Study the drawing (mm; zero at the part's minimum x, y, z) and answer. A direction names the side the tool comes from. Give positions to 0.01 mm unless a question says otherwise; leave off trailing zeros. Loops run counter-clockwise (first coordinate to the right, second up) from the corner with the lowest first, then second, coordinate; pieces in that order, holes last. Notation, with made-up numbers: M 67.5,30 L 86.5,30 A24 ccw 86.5,62 Z; hole C 25,16 d7. An arc over 180 degrees is marked long. Return JSON: item names as keys, results as strings.
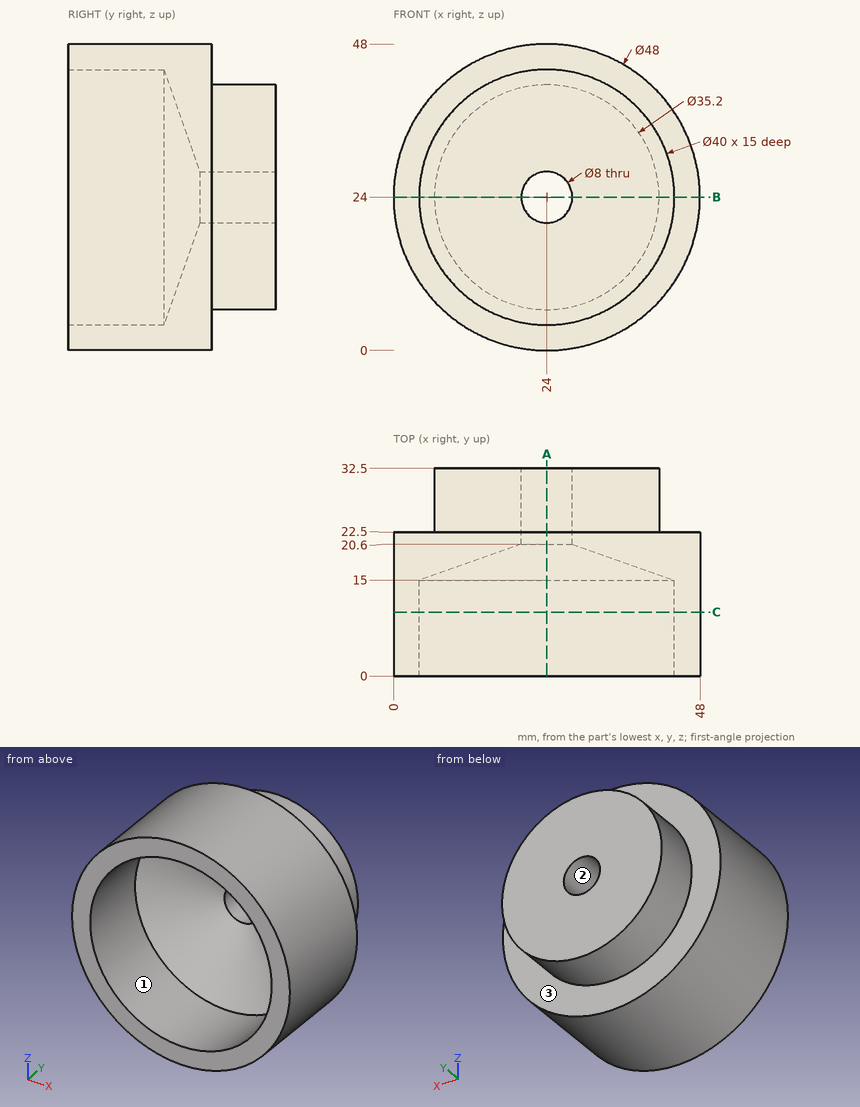
(1) The part is cut by section B-B (z = 24). Determine the outline of the cut face in (x, y), and give its area (3 significant figures).
Values follow:
{"outline": "M 0,0 L 4,0 L 4,15 L 20,20.6 L 20,32.5 L 6.4,32.5 L 6.4,22.5 L 0,22.5 Z; M 28,20.6 L 44,15 L 44,0 L 48,0 L 48,22.5 L 41.6,22.5 L 41.6,32.5 L 28,32.5 Z", "area": "602 mm²"}
(2) Given pin 1 (2 mm diameter, centred on y = 16, z = 22.5, fed in from -X); pin 2 (1 mm diameter, centred on y = 12, z = 29, fed in from +X); pin 3 (1 mm diameter, centred on x = 34, y = 8, fed in from -Z), each flat-ended and moving along its own axis, determine where each tip first touches the part or whether it passes through.
Values follow:
{"pin 1": "x = 0.01", "pin 2": "x = 47.57", "pin 3": "z = 1.96"}
(3) Straight lines are drawn through the part: line 1 along X through (y, z) = (9, 24.5); line 2 along X through (y, z) = (24.25, 24); line 3 along Y through (x, z) = (22, 4). For each, find the intervals that lie inside material, in ascending order.
Values follow:
{"line 1": "0.01 to 4.01, 43.99 to 47.99", "line 2": "6.4 to 20, 28 to 41.6", "line 3": "0 to 22.5"}
(4) The part is cut by section A-A (x = 24). Determine the outline of the cut face in (y, z).
Values follow:
{"outline": "M 0,0 L 22.5,0 L 22.5,6.4 L 32.5,6.4 L 32.5,20 L 20.6,20 L 15,4 L 0,4 Z; M 0,44 L 15,44 L 20.6,28 L 32.5,28 L 32.5,41.6 L 22.5,41.6 L 22.5,48 L 0,48 Z"}
(5) A tool of negligible diameter and unlimited length cuts with its end or side. For the marked faces 1, 2 and 3, from which of +Z, -Z, +X, -X, +Y, -Y can it reach the whole face along a straight path? Write none if from no direction.
Values follow:
{"face 1": "-Y", "face 2": "+Y, -Y", "face 3": "+Y"}
(6) The part is cut by section C-C (y = 10). Determine the outline of the cut face in (x, z).
Values follow:
{"outline": "C 24,24 d48; hole C 24,24 d40"}
